Check sheet for the modelled part. Datum: model origin and axes. Units: mm. A direction names the side the tool comes from. Round coordinates to 2 decimals unless told otherwise and drop trailing zeros. Order: outer loops, then holes, each group sorted by start corner. A loop starts at its lowest first (then second) coordinate and runs counter-clockwise, first axis right, second up. Notation, with made-up numbers: (35, 82) -> (47, 82) arc R15 cw to (47, 102) -> close; hole circle Ø8 at (-7, -7). An arc over 180 degrees is marked (long way). Answer in a Markdown table with one row per item.
```python
from build123d import *

# Parameters (mm, degrees)
SKETCH1_W           = 616
SKETCH1_H           = 35
BOSS_EXTRUDE1_DEPTH = 220
SKETCH2_W           = 153.942859838
SKETCH2_H           = 90.763998287
SKETCH2_W_2         = 159.281918562
CUT_EXTRUDE1_DEPTH  = 381.117087224


with BuildPart() as part:
    # Sketch1 → Boss-Extrude1 (new body)
    with BuildSketch(Plane(origin=(0, 0, 0), x_dir=(1, 0, 0), z_dir=(0, 1, 0))):
        Rectangle(SKETCH1_W, SKETCH1_H)
    extrude(amount=BOSS_EXTRUDE1_DEPTH)

    # Sketch2 → Cut-Extrude1 (cut, through all)
    with BuildSketch(Plane.XY.offset(17.5)):
        with Locations((-148.603801116, 124.459950708)):
            Rectangle(SKETCH2_W, SKETCH2_H)
        with Locations((138.815526791, 124.459950708)):
            Rectangle(SKETCH2_W_2, SKETCH2_H)
    extrude(amount=-CUT_EXTRUDE1_DEPTH, mode=Mode.SUBTRACT)


solid = part.part
```
(1) Section check B-B on y = 152. Record the boundary of the cut face in (x, z), plus the area to 3 significant figures.
Solutions:
| item | result |
|---|---|
| outline | (-308, -17.5) -> (-225.58, -17.5) -> (-225.58, 17.5) -> (-308, 17.5) -> close; (-71.63, -17.5) -> (59.17, -17.5) -> (59.17, 17.5) -> (-71.63, 17.5) -> close; (218.46, -17.5) -> (308, -17.5) -> (308, 17.5) -> (218.46, 17.5) -> close |
| area | 10,600 mm^2 |
(2) Section check C-C on z = -11. Record the boundary of the cut face in (x, y).
Solutions:
| item | result |
|---|---|
| outline | (-308, 0) -> (308, 0) -> (308, 220) -> (-308, 220) -> close; hole (-225.58, 79.08) -> (-71.63, 79.08) -> (-71.63, 169.84) -> (-225.58, 169.84) -> close; hole (59.17, 79.08) -> (218.46, 79.08) -> (218.46, 169.84) -> (59.17, 169.84) -> close |
(3) Draft check along X on faces 3 (the flat face through (-308, 108, 0)), 4 (the flat face through (308, 108, 0)), 5 (the flat face through (-150, 79.078, 0)). Enter one of: pulls with the +X half, pulls with the -X half, needs draft (parallel to the pull), parting line crosses it, or undercut.
Solutions:
| item | result |
|---|---|
| face 3 | pulls with the -X half |
| face 4 | pulls with the +X half |
| face 5 | undercut |
(4) Tool access check on faces 1 (the flat face through (-4, 220, 0)), 2 (the flat face through (-150, 169.842, 0)). Record the directions out of +Z, -Z, +X, -X, +Y, -Y that give a thin tool (end or side, any length) a straight path to the whole face; none if there is none.
Solutions:
| item | result |
|---|---|
| face 1 | +Z, -Z, +X, -X, +Y |
| face 2 | +Z, -Z |
(5) Section check A-A on x = -153. Record the boundary of the cut face in (y, z).
Solutions:
| item | result |
|---|---|
| outline | (0, -17.5) -> (79.08, -17.5) -> (79.08, 17.5) -> (0, 17.5) -> close; (169.84, -17.5) -> (220, -17.5) -> (220, 17.5) -> (169.84, 17.5) -> close |
(6) Scan lines: probe 1 along X at (y, z) = (147.5, -4.5); probe 2 along Y at (x, z) = (-125.5, 0). Record each from-to range of solid material in increasing order. Write a range as from..to.
Solutions:
| item | result |
|---|---|
| probe 1 | -308..-225.58, -71.63..59.17, 218.46..308 |
| probe 2 | 0..79.08, 169.84..220 |
